```python
from build123d import *

# Parameters (mm, degrees)
BRACKET_PROFILE_SKETCH_R     = 10
BRACKET_BODY_DEPTH           = 22.5
CLEVIS_SLOT_SKETCH_W         = 92
CLEVIS_SLOT_SKETCH_H         = 25
CLEVIS_SLOT_10MM_DEPTH       = 375
RELIEF_CUT_DEPTH             = 375
BODY_EDGE_CHAMFER_4MM_A_SIZE = 4
SLOT_EDGE_CHAMFER_4MM_A_SIZE = 4
BODY_EDGE_CHAMFER_4MM_B_SIZE = 4
SLOT_EDGE_CHAMFER_4MM_B_SIZE = 4
RELIEF_CUT_CHAMFER_4MM_SIZE  = 4


with BuildPart() as part:
    # Bracket Profile Sketch → Bracket Body (new, symmetric)
    with BuildSketch(Plane(origin=(0, 0, 0), x_dir=(1, 0, 0), z_dir=(0, 1, 0))):
        with BuildLine():
            Line((-33.763763442, 80.378372182), (-58.314624342, 55.827511282))
            ThreePointArc((-58.314624342, 55.827511282), (-61.158005144, 50.061705392), (-59.903810568, 43.75644347))
            Line((-59.903810568, 43.75644347), (-25.980762114, -15))
            ThreePointArc((-25.980762114, -15), (0, -30), (25.980762114, -15))
            Line((25.980762114, -15), (59.903810568, 43.75644347))
            ThreePointArc((59.903810568, 43.75644347), (61.158005144, 50.061705392), (58.314624342, 55.827511282))
            Line((58.314624342, 55.827511282), (33.763763442, 80.378372182))
            ThreePointArc((33.763763442, 80.378372182), (27.429610139, 89.711207915), (24.989530399, 100.723443462))
            ThreePointArc((24.989530399, 100.723443462), (0, 125), (-24.989530399, 100.723443462))
            ThreePointArc((-24.989530399, 100.723443462), (-27.429610139, 89.711207915), (-33.763763442, 80.378372182))
        make_face()
        with Locations(Location((0, 0, 0), (0, 0, 90))):
            Circle(BRACKET_PROFILE_SKETCH_R, mode=Mode.SUBTRACT)
        with Locations(Location((0, 100, 0), (0, 0, 90))):
            Circle(BRACKET_PROFILE_SKETCH_R, mode=Mode.SUBTRACT)
    extrude(amount=BRACKET_BODY_DEPTH, both=True)

    # Clevis Slot Sketch → Clevis Slot 10mm (cut)
    with BuildSketch(Plane(origin=(100, 0, 0), x_dir=(0, 0, -1), z_dir=(1, 0, 0))):
        with Locations((16, 0)):
            Rectangle(CLEVIS_SLOT_SKETCH_W, CLEVIS_SLOT_SKETCH_H)
    extrude(amount=-CLEVIS_SLOT_10MM_DEPTH, mode=Mode.SUBTRACT)

    # Relief Cut Sketch → Relief Cut (cut)
    with BuildSketch(Plane(origin=(100, 0, 0), x_dir=(0, 0, -1), z_dir=(1, 0, 0))):
        with BuildLine():
            Line((60, 22.5), (125, 22.5))
            Line((125, 22.5), (125, 10.5))
            Line((125, 10.5), (81.354156504, 10.5))
            ThreePointArc((81.354156504, 10.5), (69.10670779, 13.705505282), (60, 22.5))
        make_face()
        with BuildLine():
            Line((81.354156504, -10.5), (125, -10.5))
            Line((125, -10.5), (125, -22.5))
            Line((125, -22.5), (60, -22.5))
            ThreePointArc((60, -22.5), (69.10670779, -13.705505282), (81.354156504, -10.5))
        make_face()
    extrude(amount=-RELIEF_CUT_DEPTH, mode=Mode.SUBTRACT)

    # Body Edge Chamfer 4mm A
    body_edge_chamfer_4mm_a_edges = [part.edges().sort_by_distance(p)[0] for p in [
        (0, 22.5, 10),
    ]]
    chamfer(body_edge_chamfer_4mm_a_edges, length=BODY_EDGE_CHAMFER_4MM_A_SIZE)

    # Slot Edge Chamfer 4mm A
    slot_edge_chamfer_4mm_a_edges = [part.edges().sort_by_distance(p)[0] for p in [
        (0, 12.5, 10),
    ]]
    chamfer(slot_edge_chamfer_4mm_a_edges, length=SLOT_EDGE_CHAMFER_4MM_A_SIZE)

    # Body Edge Chamfer 4mm B
    body_edge_chamfer_4mm_b_edges = [part.edges().sort_by_distance(p)[0] for p in [
        (0, -22.5, 10),
    ]]
    chamfer(body_edge_chamfer_4mm_b_edges, length=BODY_EDGE_CHAMFER_4MM_B_SIZE)

    # Slot Edge Chamfer 4mm B
    slot_edge_chamfer_4mm_b_edges = [part.edges().sort_by_distance(p)[0] for p in [
        (0, -12.5, 10),
    ]]
    chamfer(slot_edge_chamfer_4mm_b_edges, length=SLOT_EDGE_CHAMFER_4MM_B_SIZE)

    # Relief Cut Chamfer 4mm
    relief_cut_chamfer_4mm_edges = [part.edges().sort_by_distance(p)[0] for p in [
        (0, 10.5, -90),
        (0, -10.5, -90),
    ]]
    chamfer(relief_cut_chamfer_4mm_edges, length=RELIEF_CUT_CHAMFER_4MM_SIZE)


solid = part.part
```
Part model, mm, in its own coordinate system. A direction names the side the tool comes from. Round coordinates to 2 decimals unless told otherwise and drop trailing zeros. Write each loop counter-clockwise with the first axis right and the second up, starting at its lowest first coordinate (ties: lowest second). Pieces come first, ordered by that corner, then holes. Notation, with made-up numbers: M 35,17.5 L 40,17.5 A29 cw 40,46.5 Z; hole C -34,4.5 d1. An arc over 180 degrees is marked long. One line per question, with ' | ' between items.
(1) 3-axis set-ups, long thin cutter, end or side, ignore diameter. For faces 4 (the face through (1, 12.5, -26)), 5 (the face through (-10.006, -16.25, 2.222)), 6 (the face through (42.705, 17.57, -13.967)): which of +Z, -Z, +X, -X, +Y, -Y reach the whole face in a straight line?
Answer key:
face 4: +Z, +X, -X | face 5: none | face 6: +Z, +X, +Y, -Y
(2) Saw through at B-B on x = -19.5. Write the cut outline in (y, z).
Answer key:
outline: M -22.5,-60 A25 cw -10.5,-81.35 L -10.5,-115.64 L 10.5,-115.64 L 10.5,-81.35 A25 cw 22.5,-60 L 22.5,22.8 L 12.5,22.8 L 12.5,-62 L -12.5,-62 L -12.5,22.8 L -22.5,22.8 Z
(3) Probe line 1 along Y through (x, z) = (-23, -8.5); line 2 along X through (y, z) = (-1.25, -100); line 3 along X through (y, z) = (-17, 0). List the from-to ranges inside material, lowest first.
Answer key:
line 1: y = -22.5 to -12.5, 12.5 to 22.5 | line 2: x = -25.02 to -10, 10 to 25.02 | line 3: x = -34.64 to -10, 10 to 34.64
(4) Two-plate mould, pull along X, no slides. Class faces 1 (the face through (-43.18, -17.43, -14.79)), 2 (the face through (42.705, -17.43, -13.967)), 3 (the face through (-3.06, -18.69, -9.72)): released by +X, released by -X, zero draft, split by the parting line, or undercut.
Answer key:
face 1: released by -X | face 2: released by +X | face 3: undercut
(5) Saw through at A-A on z = 0. Write the cut outline in (x, y).
Answer key:
outline: M -34.64,-22.5 L -14,-22.5 L -10,-18.5 L -10,-16.5 L -14,-12.5 L -34.64,-12.5 Z; M -34.64,12.5 L -14,12.5 L -10,16.5 L -10,18.5 L -14,22.5 L -34.64,22.5 Z; M 10,-18.5 L 14,-22.5 L 34.64,-22.5 L 34.64,-12.5 L 14,-12.5 L 10,-16.5 Z; M 10,16.5 L 14,12.5 L 34.64,12.5 L 34.64,22.5 L 14,22.5 L 10,18.5 Z
(6) Pin check, flat tips, straight feed: pin 1 (18 mm diameter, centred on x = 0, z = 0, fed in from +Y); pin 2 (20 mm diameter, centred on x = 24.5, y = -1, fed in from +Z); pin 3 (1 mm diameter, centred on x = 16, y = 5.5, fed in from -Z); pin 4 (1 mm diameter, centred on y = 9, z = -102, fed in from -X). Stop position of each tip, or through.
Answer key:
pin 1: passes through | pin 2: stops at z = -62 | pin 3: stops at z = -119.62 | pin 4: stops at x = -24.95
(7) Saw through at C-C on x = 0. Count the separate pieces of the cut face and the enclosed holes in it, then the cut area to 3 significant figures.
Answer key:
separate pieces: 4 | enclosed holes: 0 | area: 2,350 mm^2
(8) Saw through at D-D on z = -64.5. Write the cut outline in (x, y).
Answer key:
outline: M -49.64,-17.04 L 49.64,-17.04 L 49.64,17.04 L -49.64,17.04 Z
